```python
from build123d import *

# Parameters (mm, degrees)
BASE_ARM_8MM_DEPTH   = 4
FINGER_SLOTS_DEPTH   = 8
SIDE_SLOT_PROFILE_R  = 0.7
SIDE_SLOT_DEPTH      = 12.515344682
CLEVIS_LUG_8MM_DEPTH = 4
LUG_END_ROUND_R4_R   = 4
EDGE_FILLET_R0_4_R   = 0.4
LUG_FILL_BOSS_DEPTH  = 1.8
LUG_BLEND_BOSS_DEPTH = 1.6
PIN_HOLE_PROFILE_R   = 1.6
PIN_HOLE_3_2_DEPTH   = 13.647446253


with BuildPart() as part:
    # Base Arm Profile → Base Arm 8mm (new, symmetric)
    with BuildSketch(Plane.XY):
        Polygon((0, 0), (-7.356734921, -6.3951121), (-8.668852979, -4.88569294), (-1.876466757, 1.018838321), (-1.041428151, 6.960446733), (0.939107986, 6.682100531), align=None)
    extrude(amount=BASE_ARM_8MM_DEPTH, both=True)

    # Finger Slots Profile → Finger Slots (cut)
    with BuildSketch(Plane(origin=(-1.980536137, 0.278346202, 0), x_dir=(0, 0, 1), z_dir=(-0.9902680687415697, 0.13917310096006985, 0))):
        with BuildLine():
            Line((-2.7, 4.747769359), (-2.7, 6.747769359))
            Line((-2.7, 6.747769359), (-1.3, 6.747769359))
            Line((-1.3, 6.747769359), (-1.3, 4.747769359))
            ThreePointArc((-1.3, 4.747769359), (-2, 4.047769359), (-2.7, 4.747769359))
        make_face()
        with BuildLine():
            Line((1.3, 6.747769359), (1.3, 4.747769359))
            ThreePointArc((1.3, 4.747769359), (2, 4.047769359), (2.7, 4.747769359))
            Line((2.7, 4.747769359), (2.7, 6.747769359))
            Line((2.7, 6.747769359), (1.3, 6.747769359))
        make_face()
    extrude(amount=-FINGER_SLOTS_DEPTH, mode=Mode.SUBTRACT)

    # Side Slot Profile → Side Slot (cut, through all)
    with BuildSketch(Plane(origin=(-1.312118058, 1.50941916, 0), x_dir=(0.7547095802227755, 0.6560590289905035, 0), z_dir=(-0.6560590289905035, 0.7547095802227755, 0))):
        with Locations(Location((-7.747769359, -2, 0), (0, 0, 180))):
            Circle(SIDE_SLOT_PROFILE_R)
        with Locations(Location((-7.747769359, 2, 0), (0, 0, 180))):
            Circle(SIDE_SLOT_PROFILE_R)
    extrude(amount=-SIDE_SLOT_DEPTH, mode=Mode.SUBTRACT)

    # Clevis Lug Profile → Clevis Lug 8mm (add, symmetric)
    with BuildSketch(Plane.XY):
        Polygon((-3.681178903, -3.2), (4.123533243, -3.2), (4.123533243, -1.4), (0.939107986, -1.4), (0.939107986, 0.3), (4.123533243, 0.3), (4.123533243, 1.9), (0.267027586, 1.9), (0, 0), align=None)
    extrude(amount=CLEVIS_LUG_8MM_DEPTH, both=True)

    # Lug End Round R4
    lug_end_round_r4_edges = [part.edges().sort_by_distance(p)[0] for p in [
        (-3.681178903, -3.2, 0),
    ]]
    fillet(lug_end_round_r4_edges, radius=LUG_END_ROUND_R4_R)

    # Edge Fillet R0.4
    edge_fillet_r0_4_edges = [part.edges().sort_by_distance(p)[0] for p in [
        (0.267027586, 1.9, 0),
    ]]
    fillet(edge_fillet_r0_4_edges, radius=EDGE_FILLET_R0_4_R)

    # Lug Fill Boss Profile → Lug Fill Boss (add)
    with BuildSketch(Plane(origin=(0, -1.4, 0), x_dir=(1, 0, 0), z_dir=(0, 1, 0))):
        with BuildLine():
            Line((4.123533243, 4), (4.123533243, -4))
            ThreePointArc((4.123533243, -4), (8.123533243, 0), (4.123533243, 4))
        make_face()
    extrude(amount=-LUG_FILL_BOSS_DEPTH)

    # Lug Blend Boss Profile → Lug Blend Boss (add)
    with BuildSketch(Plane(origin=(0, 1.9, 0), x_dir=(1, 0, 0), z_dir=(0, 1, 0))):
        with BuildLine():
            Line((4.123533243, 4), (4.123533243, -4))
            ThreePointArc((4.123533243, -4), (8.123533243, 0), (4.123533243, 4))
        make_face()
    extrude(amount=-LUG_BLEND_BOSS_DEPTH)

    # Pin Hole Profile → Pin Hole Ø3.2 (cut, through all)
    with BuildSketch(Plane(origin=(0, 1.9, 0), x_dir=(1, 0, 0), z_dir=(0, 1, 0))):
        with Locations(Location((4.123533243, 0, 0), (0, 0, 180))):
            Circle(PIN_HOLE_PROFILE_R)
    extrude(amount=-PIN_HOLE_3_2_DEPTH, mode=Mode.SUBTRACT)


solid = part.part
```
Check sheet for the modelled part. Datum: model origin and axes. Units: mm. A direction names the side the tool comes from. Round coordinates to 2 decimals unless told otherwise and drop trailing zeros. Loops run counter-clockwise (first coordinate to the right, second up) from the corner with the lowest first, then second, coordinate; pieces in that order, holes last. Notation, with made-up numbers: (-8.75, 86.5) - (46.25, 86.5) arc R23 cw to (46.25, 117.5) - close; hole circle Ø11 at (-32, -8). An arc over 180 degrees is marked (long way). Write item = value, one per line. Start each with the question number.
Q1. Section check C-C (x = 6.25). Record the boundary of the cut face in (y, z).
Q2. Depth check by flat-ended pin: P1, Ø3.5, axis at x = 5, z = 0.5, coming from the -Y side; P2, Ø0.5, axis at y = -1, z = 1, coming from the +X side; P3, Ø1, axis at x = -4.5, z = -1, coming from the -Y side. Enter the tip coordinate at first touch or a pass-through.
Q3. Section check D-D (z = 3). Record the boundary of the cut face in (x, y), plus the area to 3 significant figures.
Q4. Section check A-A (x = 1.25). Record the boundary of the cut face in (y, z).
Q5. Section check B-B (z = 0). Record the boundary of the cut face in (x, y).
Q6. Release check for a two-part mould opening along Y. For faces 1 (the face through (4, 0.3, -2)), 2 (the face through (0, 6, 2.7)), 3 (the face through (-1.465, 3.948, 0.056)) record: pulls with the +Y half, pulls with the -Y half, needs draft (parallel to the pull), parting line crosses it, or undercut.
Q7. Access from +Z, -Z, +X, -X, +Y, -Y to the whole of each face (thin tool, end or side, straight path). Record for faces 4 (the face through (-0.44, 4.15, 1.98)), 5 (the face through (0.64, 4.55, 0.06)).
Q8. Thickness scan on L1, parallel to Y at x = 1.75, z = -1.5; L2, parallel to Z at x = -6.5, y = -3.75; L3, parallel to Z at x = 4.75, y = 1.75. Record the ranges inside material, lowest first.
Derived:
q1.outline = (-3.2, -3.39) - (-1.4, -3.39) - (-1.4, 3.39) - (-3.2, 3.39) - close; (0.3, -3.39) - (1.9, -3.39) - (1.9, 3.39) - (0.3, 3.39) - close
q2.P1 = -3.2
q2.P2 = 0.94
q2.P3 = -4.35
q3.outline = (-8.67, -4.89) - (-7.36, -6.4) - (-4.81, -4.18) arc R4 cw to (-2.19, -3.2) - (6.77, -3.2) - (6.77, -1.4) - (0.94, -1.4) - (0.94, 0.3) - (6.77, 0.3) - (6.77, 1.9) - (0.73, 1.9) arc R0.4 cw to (0.33, 2.36) - (0.94, 6.68) - (-1.04, 6.96) - (-1.88, 1.02) - close
q3.area = 62.0 mm^2
q4.outline = (-3.2, -4) - (-1.4, -4) - (-1.4, 4) - (-3.2, 4) - close; (0.3, -4) - (1.9, -4) - (1.9, 4) - (0.3, 4) - close
q5.outline = (-8.67, -4.89) - (-7.36, -6.4) - (-4.81, -4.18) arc R4 cw to (-2.19, -3.2) - (2.52, -3.2) - (2.52, -1.4) - (0.94, -1.4) - (0.94, 0.3) - (2.52, 0.3) - (2.52, 1.9) - (0.73, 1.9) arc R0.4 cw to (0.33, 2.36) - (0.94, 6.68) - (-1.04, 6.96) - (-1.88, 1.02) - close; (5.72, -3.2) - (8.12, -3.2) - (8.12, -1.4) - (5.72, -1.4) - close; (5.72, 0.3) - (8.12, 0.3) - (8.12, 1.9) - (5.72, 1.9) - close
q6.face_1 = undercut
q6.face_2 = needs draft
q6.face_3 = pulls with the +Y half
q7.face_4 = +X, +Y
q7.face_5 = +Z, -Z, +X
q8.L1 = -3.2 to -1.4, 0.3 to 1.9
q8.L2 = -4 to -2.59, -1.41 to 1.41, 2.59 to 4
q8.L3 = -3.95 to -1.47, 1.47 to 3.95
